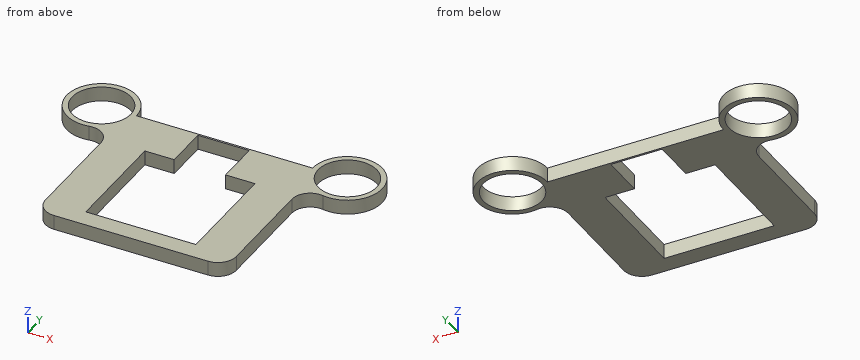
```python
from build123d import *

# Parameters (mm, degrees)
SKETCH_1_R      = 16
EXTRUDE_1_DEPTH = 8


with BuildPart() as part:
    # 草图1 → 凸台-拉伸1 (new body)
    with BuildSketch(Plane.XY):
        with BuildLine():
            ThreePointArc((63.331817296, 16.731279855), (81.154867742, 47.668830358), (47.607679365, 35.446747461))
            Line((47.607679365, 35.446747461), (-47.607679365, 35.446747461))
            Line((-47.607679365, 35.446747461), (-48.392320635, 35.446747461))
            ThreePointArc((-48.392320635, 35.446747461), (-81.939509011, 47.668830358), (-64.116458566, 16.731279855))
            ThreePointArc((-64.116458566, 16.731279855), (-55.959645426, 14.537448682), (-52.392320635, 6.881033747))
            Line((-52.392320635, 6.881033747), (-52.392320635, -49.553252539))
            ThreePointArc((-52.392320635, -49.553252539), (-49.463388447, -56.624320351), (-42.392320635, -59.553252539))
            Line((-42.392320635, -59.553252539), (41.607679365, -59.553252539))
            ThreePointArc((41.607679365, -59.553252539), (48.678747177, -56.624320351), (51.607679365, -49.553252539))
            Line((51.607679365, -49.553252539), (51.607679365, 6.881033747))
            ThreePointArc((51.607679365, 6.881033747), (55.175004156, 14.537448682), (63.331817296, 16.731279855))
        make_face()
        Polygon((19.522836201, -49.553252539), (-28.363655741, -49.553252539), (-30.392320635, -49.553252539), (-30.392320635, 10.446747461), (-14.392320635, 10.446747461), (-14.392320635, 34.446747461), (13.607679365, 34.446747461), (13.607679365, 10.446747461), (29.607679365, 10.446747461), (29.607679365, -49.553252539), align=None, mode=Mode.SUBTRACT)
        with Locations((-67.392320635, 35.446747461)):
            Circle(SKETCH_1_R, mode=Mode.SUBTRACT)
        with Locations((66.607679365, 35.446747461)):
            Circle(SKETCH_1_R, mode=Mode.SUBTRACT)
    extrude(amount=EXTRUDE_1_DEPTH)


solid = part.part
```
CAD build for the part. Positions are in the model's coordinates, mm. Round coordinates to 2 decimals unless told otherwise and drop trailing zeros. Order: outer loops, then holes, each group sorted by start corner. A loop starts at its lowest first (then second) coordinate and runs counter-clockwise, first axis right, second up. Notation, with made-up numbers: (61, 14.25) - (90, 14.25) arc R21 ccw to (90, 42.25) - close; hole circle Ø9 at (-35, 11). An arc over 180 degrees is marked (long way). Answer in a Markdown table with one row per item. Add a question column.
(1) Band-saw the part on A-A on y = -13. List the corners of the cut face in (x, z), and give its area (3 significant figures).
(2) Band-saw the part on C-C on y = 47. List the corners of the cut face in (x, z), and give its area (3 significant figures).
(3) Band-saw the part on D-D on z = 5.25. List the corners of the cut face in (x, y), and give its area (3 significant figures).
(4) Probe L1, parallel to X at y = -20, z = 3.5; L2, parallel to Y at x = 16, z = 3.5; L3, parallel to X at y = 27.5, z = 2. List the from-to ranges inside material, lowest first. Write a range as [from, to].
(5) Band-saw the part on B-B on x = -5.5. List the corners of the cut face in (y, z).
(6) Drop flat-ended pins along their axis: pin 1 Ø6 at (x, y) = (-11.5, 7.5) entering from +Z; pin 2 Ø2.5 at (y, z) = (19, 5.5) entering from +X; pin 3 Ø2.5 at (y, z) = (-22, 2.5) entering from -X; pin 4 Ø4 at (y, z) = (22, 2.5) entering from -X. Give the stop position or say it passes through.
Data:
| question | item | result |
|---|---|---|
| 1 | outline | (-52.39, 0) - (-30.39, 0) - (-30.39, 8) - (-52.39, 8) - close; (29.61, 0) - (51.61, 0) - (51.61, 8) - (29.61, 8) - close |
| 1 | area | 352 mm^2 |
| 2 | outline | (-82.48, 0) - (-78.46, 0) - (-78.46, 8) - (-82.48, 8) - close; (-56.32, 0) - (-52.31, 0) - (-52.31, 8) - (-56.32, 8) - close; (51.52, 0) - (55.54, 0) - (55.54, 8) - (51.52, 8) - close; (77.68, 0) - (81.69, 0) - (81.69, 8) - (77.68, 8) - close |
| 2 | area | 128 mm^2 |
| 3 | outline | (-64.12, 16.73) arc R10 cw to (-52.39, 6.88) - (-52.39, -49.55) arc R10 ccw to (-42.39, -59.55) - (41.61, -59.55) arc R10 ccw to (51.61, -49.55) - (51.61, 6.88) arc R10 cw to (63.33, 16.73) arc R19 ccw (long way) to (47.61, 35.45) - (-48.39, 35.45) arc R19 ccw (long way) to start; hole circle Ø32 at (-67.39, 35.45); hole (-30.39, -49.55) - (29.61, -49.55) - (29.61, 10.45) - (13.61, 10.45) - (13.61, 34.45) - (-14.39, 34.45) - (-14.39, 10.45) - (-30.39, 10.45) - close; hole circle Ø32 at (66.61, 35.45) |
| 3 | area | 6,260 mm^2 |
| 4 | L1 | x = [-52.39, -30.39], [29.61, 51.61] |
| 4 | L2 | y = [-59.55, -49.55], [10.45, 35.45] |
| 4 | L3 | x = [-84.65, -81.28], [-53.51, -14.39], [13.61, 52.72], [80.49, 83.87] |
| 5 | outline | (-59.55, 0) - (-49.55, 0) - (-49.55, 8) - (-59.55, 8) - close; (34.45, 0) - (35.45, 0) - (35.45, 8) - (34.45, 8) - close |
| 6 | pin 1 | passes through |
| 6 | pin 2 | stops at x = 78.01 |
| 6 | pin 3 | stops at x = -52.39 |
| 6 | pin 4 | stops at x = -82.56 |
